Print and shaded views of the part. All mm, measured from the part's lowest x, y and z. Give positions to 0.01 mm unless a question says otherwise; leave off trailing zeros. Loops run counter-clockwise (first coordinate to the right, second up) from the corner with the lowest first, then second, coordinate; pieces in that order, holes last. Notation, with made-up numbers: (15, 76) -> (31, 76) arc R17 ccw to (31, 106) -> close; hole circle Ø2 at (78.5, 6). An arc over 180 degrees is marked (long way). Write each question's results on one line, items separated by ' | '. Start each with the question number.
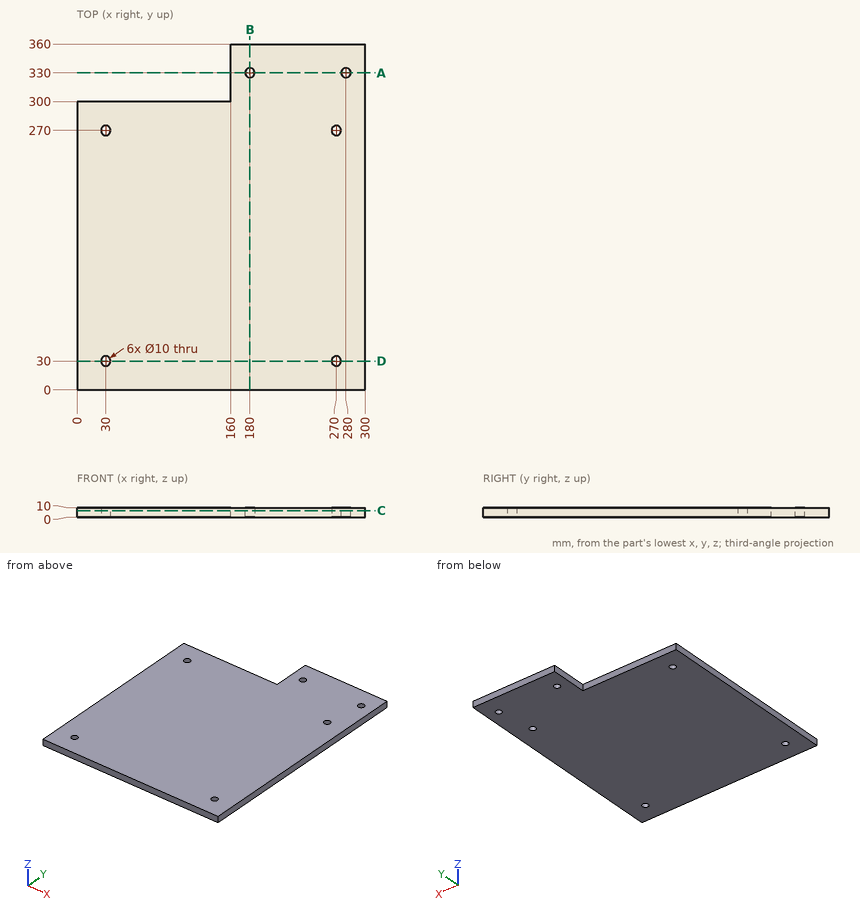
Q1. Drop flat-ended pins along their axis: pin 1 (5 mm diameter, centred on x = 70.5, z = 3.5, fed in from +Y); pin 2 (6 mm diameter, centred on x = 280, y = 330, fed in from -Z) (3 decimals). Give the stop position or say it passes through.
Q2. Saw through at A-A, the plane y = 330. List the corners of the cut face in (x, z), then the cut area to 3 significant figures.
Q3. Saw through at D-D, the plane y = 30. List the corners of the cut face in (x, z), then the cut area to 3 significant figures.
Q4. Saw through at B-B, the plane x = 180. List the corners of the cut face in (y, z).
Q5. Saw through at C-C, the plane z = 7. List the corners of the cut face in (x, y).
Q6. Wall check: L1, parallel to Y at x = 270, z = 3.5; L2, parallel to Y at x = 180, z = 6; L3, parallel to X at y = 270, z = 7.25. Give the ranges that are in metal, low to high.
Answer block:
1) pin 1: stops at y = 300 | pin 2: passes through
2) outline: (160, 0) -> (175, 0) -> (175, 10) -> (160, 10) -> close; (185, 0) -> (275, 0) -> (275, 10) -> (185, 10) -> close; (285, 0) -> (300, 0) -> (300, 10) -> (285, 10) -> close | area: 1,200 mm2
3) outline: (0, 0) -> (25, 0) -> (25, 10) -> (0, 10) -> close; (35, 0) -> (265, 0) -> (265, 10) -> (35, 10) -> close; (275, 0) -> (300, 0) -> (300, 10) -> (275, 10) -> close | area: 2,800 mm2
4) outline: (0, 0) -> (325, 0) -> (325, 10) -> (0, 10) -> close; (335, 0) -> (360, 0) -> (360, 10) -> (335, 10) -> close
5) outline: (0, 0) -> (300, 0) -> (300, 360) -> (160, 360) -> (160, 300) -> (0, 300) -> close; hole circle Ø10 at (30, 30); hole circle Ø10 at (30, 270); hole circle Ø10 at (180, 330); hole circle Ø10 at (270, 30); hole circle Ø10 at (270, 270); hole circle Ø10 at (280, 330)
6) L1: y = 0 to 25, 35 to 265, 275 to 360 | L2: y = 0 to 325, 335 to 360 | L3: x = 0 to 25, 35 to 265, 275 to 300
